Build history of the part. All positions in model axes, mm. A direction names the side the tool comes from. Give positions to 0.01 mm unless a question says otherwise; leave off trailing zeros. Write each loop counter-clockwise with the first axis right and the second up, starting at its lowest first coordinate (ties: lowest second). Pieces come first, ordered by that corner, then holes. Notation, with made-up numbers: (17, -26.75) -> (35, -26.75) arc R9 cw to (35, -22.75) -> close; hole circle Ø3 at (-1.75, -19). An arc over 180 degrees is marked (long way). Put each result on its own line as item: value. Start each with the question number.
Item 1: Two-plate mould, pull along Y, no slides. Class faces 3 (the flat face through (-110, 140, 54)), 4 (the cylindrical face through (-104.93, 321.63, 41.68)), 5 (the flat face through (-100, 298, 54)), 6 (the cylindrical face through (-115.07, 320.346, 43.951)): pulls with the +Y half, pulls with the -Y half, needs draft (parallel to the pull), parting line crosses it, or undercut.
Item 2: Slice it at A-A, the plane y = 327. List the corners of the cut face in (x, z), plus the area to 3 significant figures.
Item 3: Flat gauge pins, fed straight in: pin 1 Ø4.5 at (y, z) = (324, 38.5) entering from -X; pin 2 Ø7.5 at (y, z) = (327.5, 91) entering from -X. Where does each tip first touch, or does it go through?
Item 4: Tool access for faces 1 (the flat face through (-110, 302, 0)), 2 (the cylindrical face through (-115.07, 319.68, 63.86)): list every direction of +Z, -Z, +X, -X, +Y, -Y with a clear straight run to the whole face (end or side of a thin tool).
Item 5: Drill centre lines: line 1 along Z through (x, y) = (-116.5, 327); line 2 along Z through (x, y) = (-107.25, 327); line 3 along Y through (x, z) = (-118.75, 91.5). Where is each one in solid material? Low to high.
Item 6: Slice it at B-B, the plane z = 65.49. List the corners of the cut face in (x, y).
Item 7: Slice it at C-C, the plane x = -115.25. List the corners of the cut face in (y, z).
```python
from build123d import *

# Parameters (mm, degrees)
SKETCH1_W                                = 20
SKETCH1_H                                = 320
BOSS_EXTRUDE1_DEPTH                      = 110
CBORE_FOR_M10_HEX_HEAD_BOLT1_D           = 11
CBORE_FOR_M10_HEX_HEAD_BOLT1_DEPTH       = 22.25
CBORE_FOR_M10_HEX_HEAD_BOLT1_CBORE_D     = 15
CBORE_FOR_M10_HEX_HEAD_BOLT1_CBORE_DEPTH = 10
CBORE_FOR_M10_HEX_HEAD_BOLT1_TIP         = 3.304733405


with BuildPart() as part:
    # Sketch1 → Boss-Extrude1 (new body)
    with BuildSketch(Plane.XY):
        with Locations((-110, 300)):
            Rectangle(SKETCH1_W, SKETCH1_H)
    extrude(amount=BOSS_EXTRUDE1_DEPTH)

    # CBORE for M10 Hex Head Bolt1
    with Locations(Plane.ZY.offset(120)):
        with Locations((40.49, 327), (65.49, 327), (90.49, 327)):
            CounterBoreHole(CBORE_FOR_M10_HEX_HEAD_BOLT1_D / 2, CBORE_FOR_M10_HEX_HEAD_BOLT1_CBORE_D / 2, CBORE_FOR_M10_HEX_HEAD_BOLT1_CBORE_DEPTH, depth=CBORE_FOR_M10_HEX_HEAD_BOLT1_DEPTH)
            with Locations((0, 0, -(CBORE_FOR_M10_HEX_HEAD_BOLT1_DEPTH + CBORE_FOR_M10_HEX_HEAD_BOLT1_TIP / 2))):  # 118° drill point
                Cone(0, CBORE_FOR_M10_HEX_HEAD_BOLT1_D / 2, CBORE_FOR_M10_HEX_HEAD_BOLT1_TIP, mode=Mode.SUBTRACT)


solid = part.part
```
Values follow:
1. face 3: pulls with the -Y half
1. face 4: undercut
1. face 5: needs draft
1. face 6: undercut
2. outline: (-120, 0) -> (-100, 0) -> (-100, 34.99) -> (-110, 34.99) -> (-110, 32.99) -> (-120, 32.99) -> close; (-120, 47.99) -> (-110, 47.99) -> (-110, 45.99) -> (-100, 45.99) -> (-100, 59.99) -> (-110, 59.99) -> (-110, 57.99) -> (-120, 57.99) -> close; (-120, 72.99) -> (-110, 72.99) -> (-110, 70.99) -> (-100, 70.99) -> (-100, 84.99) -> (-110, 84.99) -> (-110, 82.99) -> (-120, 82.99) -> close; (-120, 97.99) -> (-110, 97.99) -> (-110, 95.99) -> (-100, 95.99) -> (-100, 110) -> (-120, 110) -> close
2. area: 1,420 mm2
3. pin 1: x = -110
3. pin 2: through
4. face 1: -Z, +X, -X, +Y, -Y
4. face 2: -X
5. line 1: 0 to 32.99, 47.99 to 57.99, 72.99 to 82.99, 97.99 to 110
5. line 2: 0 to 34.99, 45.99 to 59.99, 70.99 to 84.99, 95.99 to 110
5. line 3: 140 to 319.57, 334.43 to 460
6. outline: (-120, 140) -> (-100, 140) -> (-100, 321.5) -> (-110, 321.5) -> (-110, 319.5) -> (-120, 319.5) -> close; (-120, 334.5) -> (-110, 334.5) -> (-110, 332.5) -> (-100, 332.5) -> (-100, 460) -> (-120, 460) -> close
7. outline: (140, 0) -> (460, 0) -> (460, 110) -> (140, 110) -> close; hole circle Ø15 at (327, 40.49); hole circle Ø15 at (327, 65.49); hole circle Ø15 at (327, 90.49)
